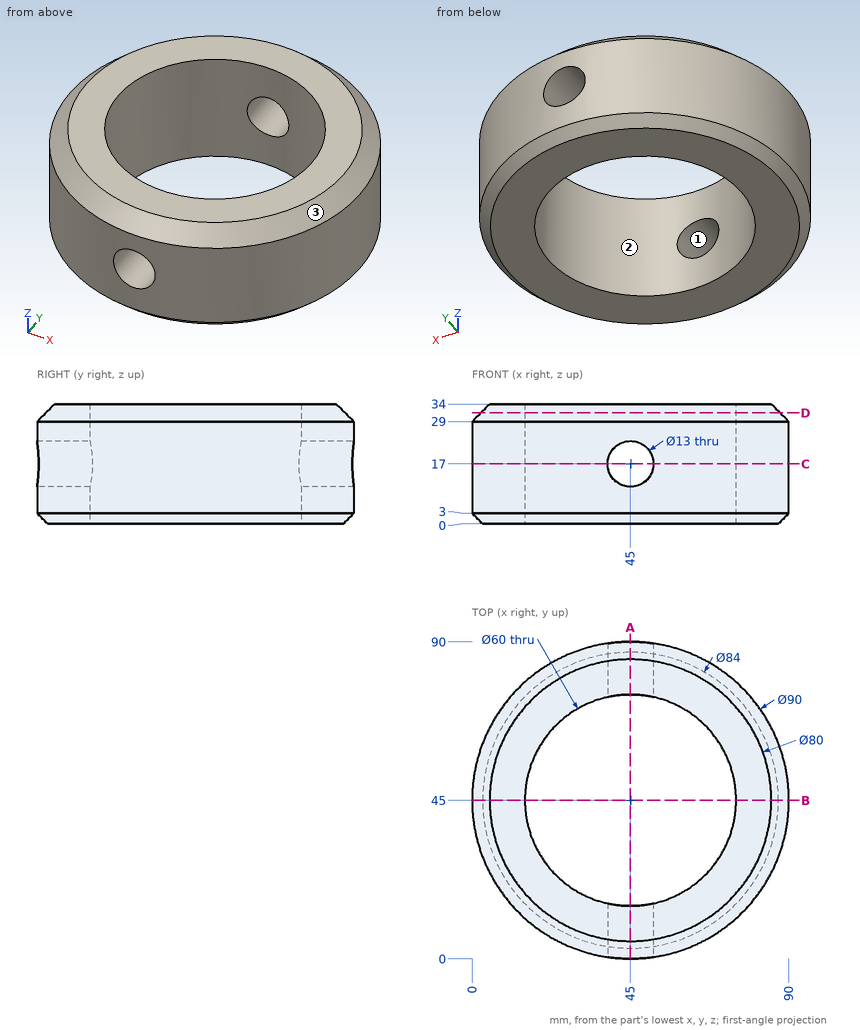
Here's the drawing with two shaded views (mm, measured from the low corner). I have some questions. Give positions to 0.01 mm unless a question says otherwise; leave off trailing zeros. Loops run counter-clockwise (first coordinate to the right, second up) from the corner with the lowest first, then second, coordinate; pieces in that order, holes last. Notation, with made-up numbers: M 40.5,-38 L 48.5,-38 A8 ccw 48.5,-32 Z; hole C -24.75,21.25 d4. An arc over 180 degrees is marked long. One line per item, written item: value.
(1) I need wall thicknesses on line 1 (Y direction, x = 45, z = 27); line 2 (X direction, y = 50, z = 28); line 3 (Y direction, x = 58, z = 7.5). Which ranges of each line are inside material? Lowest first, please.
Returned:
line 1: 0 to 15, 75 to 90
line 2: 0.28 to 15.42, 74.58 to 89.72
line 3: 1.92 to 17.96, 72.04 to 88.08
(2) We'd pull the mould along Y, two halves only. Please class the marked faces 1, 2 and 3: released by +Y, released by -Y, zero draft, split by the parting line, or undercut.
Returned:
face 1: zero draft
face 2: undercut
face 3: split by the parting line
(3) Suppose I cut it at D-D on z = 31.5. List the corners of the cut face in (x, y) for me, plus the area to 3 significant figures.
Returned:
outline: C 45,45 d85; hole C 45,45 d60
area: 2,850 mm^2
(4) Suppose I cut it at B-B on y = 45. List the corners of the cut face in (x, z) for me, plus the area to 3 significant figures.
Returned:
outline: M 0,3 L 3,0 L 15,0 L 15,34 L 5,34 L 0,29 Z; M 75,0 L 87,0 L 90,3 L 90,29 L 85,34 L 75,34 Z
area: 986 mm^2
(5) Will these pins go through, and if not, where does the flat tip stop? pin 1 (1.5 mm diameter, centred on x = 35, z = 23.5, fed in from -Y); pin 2 (2 mm diameter, centred on x = 13, z = 8.5, fed in from +Y); pin 3 (8 mm diameter, centred on x = 66, z = 26, fed in from +Y).
Returned:
pin 1: y = 0.96
pin 2: y = 77.62
pin 3: y = 86.67
(6) Suppose I cut it at C-C on z = 17. List the corners of the cut face in (x, y) for me.
Returned:
outline: M 38.5,0.47 L 38.5,15.71 A30 cw 38.5,74.29 L 38.5,89.53 A45 ccw Z; M 51.5,0.47 A45 ccw 51.5,89.53 L 51.5,74.29 A30 cw 51.5,15.71 Z
(7) Suppose I cut it at A-A on x = 45. List the corners of the cut face in (y, z) for me.
Returned:
outline: M 0,3 L 3,0 L 15,0 L 15,10.5 L 0,10.5 Z; M 0,23.5 L 15,23.5 L 15,34 L 5,34 L 0,29 Z; M 75,0 L 87,0 L 90,3 L 90,10.5 L 75,10.5 Z; M 75,23.5 L 90,23.5 L 90,29 L 85,34 L 75,34 Z
